The listing builds one solid part. Answer for the finished solid, in the listing's coordinates (mm). Face numbers are marked on the shaded views. Give positions to 0.01 mm unless a question says otherwise; leave off trailing zeros. Order: outer loops, then holes, each group sorted by start corner. A loop starts at its lowest first (then second) coordinate and runs counter-clockwise, first axis right, second up. Notation, with made-up numbers: (40.25, -1.75) -> (56.25, -1.75) arc R21 cw to (56.25, 35.25) -> close; hole circle Ø4 at (16, 30.25). An arc over 180 degrees is marked (long way). One line per question, with ' | ' between items. Start each with the question number.
```python
from build123d import *

# Parameters (mm, degrees)
JAW_PROFILE_SKETCH_R = 4
JAW_BODY_25MM_DEPTH  = 12.5
SLOT_SKETCH_W        = 25.15
SLOT_SKETCH_H        = 5
SLOT_CUT_5MM_DEPTH   = 25
EDGE_FILLETS_R1_R    = 1


with BuildPart() as part:
    # Jaw Profile Sketch → Jaw Body 25mm (new, symmetric)
    with BuildSketch(Plane.XY):
        with BuildLine():
            Line((24.825451548, -2.87524489), (45.715451548, 51.36475511))
            ThreePointArc((45.715451548, 51.36475511), (41.12524489, 61.705451548), (30.784548452, 57.11524489))
            Line((30.784548452, 57.11524489), (11.868297239, 8))
            Line((11.868297239, 8), (-17.36, 8))
            ThreePointArc((-17.36, 8), (-25.36, 0), (-17.36, -8))
            Line((-17.36, -8), (17.36, -8))
            ThreePointArc((17.36, -8), (21.887584393, -6.595527239), (24.825451548, -2.87524489))
        make_face()
        with Locations((38.25, 54.24)):
            Circle(JAW_PROFILE_SKETCH_R, mode=Mode.SUBTRACT)
        with Locations((-17.36, 0)):
            Circle(JAW_PROFILE_SKETCH_R, mode=Mode.SUBTRACT)
        with Locations((17.36, 0)):
            Circle(JAW_PROFILE_SKETCH_R, mode=Mode.SUBTRACT)
    extrude(amount=JAW_BODY_25MM_DEPTH, both=True)

    # Slot Sketch → Slot Cut 5mm (cut)
    with BuildSketch(Plane(origin=(0, 8, 0), x_dir=(1, 0, 0), z_dir=(0, 1, 0))):
        with Locations((-12.785, 0)):
            Rectangle(SLOT_SKETCH_W, SLOT_SKETCH_H)
    extrude(amount=-SLOT_CUT_5MM_DEPTH, mode=Mode.SUBTRACT)

    # Edge Fillets R1
    edge_fillets_r1_edges = [part.edges().sort_by_distance(p)[0] for p in [
        (11.868297239, 8, 0),
    ]]
    fillet(edge_fillets_r1_edges, radius=EDGE_FILLETS_R1_R)


solid = part.part
```
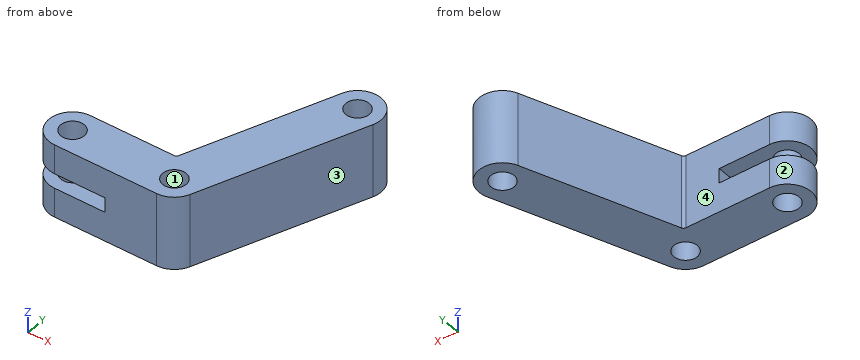
(1) Given P1, Ø8, axis at x = -18, y = -2.5, coming from the -Z side; P2, Ø5, axis at y = 51.5, z = 1.5, coming from the +X side; P3, Ø12, axis at y = 44, z = 0.5, coming from the +X side; P4, Ø4, axis at x = 5, z = -2, coming from the +Y side, each flat-ended and moving along its own axis, determine where each tip first touches the part or whether it passes through.
(2) The part is cut by section B-B on x = 38.5. Determine the outline of the cut face in (y, z).
(3) The part is cut by section C-C on y = 0. Determine the outline of the cut face in (x, z).
(4) Determine the mould class of the marked faces 1, 2, 3 and 4 for opening direction Y: pulls with the +Y half, pulls with the -Y half, needs draft (parallel to the pull), parting line crosses it, or undercut.
(5) The part is cut by section A-A on z = 8.5. Determine the outline of the cut face in (x, y), plus the area to 3 significant figures.
(6) Consider line 1 (Z direction, x = -7, y = 7.5); line 2 (Y direction, x = -17.36, z = -7.75); line 3 (X direction, y = -3.5, z = -7.75). Determine where each line is inside the solid, lowest interval first.
(7) The part is cut by section D-D on z = 0. Determine the outline of the cut face in (x, y), plus the area to 3 significant figures.
Result sheet:
1) P1: stops at z = -12.5 | P2: stops at x = 46.25 | P3: stops at x = 45.19 | P4: stops at y = 8
2) outline: (32.63, -12.5) -> (50.25, -12.5) -> (50.25, 12.5) -> (32.63, 12.5) -> close; (58.23, -12.5) -> (62.24, -12.5) -> (62.24, 12.5) -> (58.23, 12.5) -> close
3) outline: (-25.36, -12.5) -> (-21.36, -12.5) -> (-21.36, -2.5) -> (-25.36, -2.5) -> close; (-25.36, 2.5) -> (-21.36, 2.5) -> (-21.36, 12.5) -> (-25.36, 12.5) -> close; (-13.36, -12.5) -> (13.36, -12.5) -> (13.36, 12.5) -> (-13.36, 12.5) -> (-13.36, 2.5) -> (-0.21, 2.5) -> (-0.21, -2.5) -> (-13.36, -2.5) -> close; (21.36, -12.5) -> (25.93, -12.5) -> (25.93, 12.5) -> (21.36, 12.5) -> close
4) face 1: undercut | face 2: parting line crosses it | face 3: pulls with the -Y half | face 4: pulls with the +Y half
5) outline: (-17.36, -8) -> (17.36, -8) arc R8 ccw to (24.83, -2.88) -> (45.72, 51.36) arc R8 ccw to (30.78, 57.12) -> (12.12, 8.64) arc R1 cw to (11.18, 8) -> (-17.36, 8) arc R8 ccw to start; hole circle Ø8 at (-17.36, 0); hole circle Ø8 at (17.36, 0); hole circle Ø8 at (38.25, 54.24) | area: 1,530 mm^2
6) line 1: z = -12.5 to -2.5, 2.5 to 12.5 | line 2: y = -8 to -4, 4 to 8 | line 3: x = -24.55 to -19.3, -15.42 to 15.42, 19.3 to 24.55
7) outline: (-0.21, -8) -> (17.36, -8) arc R8 ccw to (24.83, -2.88) -> (45.72, 51.36) arc R8 ccw to (30.78, 57.12) -> (12.12, 8.64) arc R1 cw to (11.18, 8) -> (-0.21, 8) -> close; hole circle Ø8 at (17.36, 0); hole circle Ø8 at (38.25, 54.24) | area: 1,210 mm^2
